Geometry: final body of the model. Coordinates: model frame, mm. A direction names the side the tool comes from. Give positions to 0.01 mm unless a question says otherwise; leave off trailing zeros. Loops run counter-clockwise (first coordinate to the right, second up) from the corner with the lowest first, then second, coordinate; pieces in that order, holes last. Notation, with made-up numbers: (3.5, 22.25) - (10.5, 22.25) arc R22 ccw to (10.5, 35.25) - close; hole circle Ø10 at (52, 49.25). An arc over 180 degrees is marked (long way). Use CSV: the item, a comma, the result in double quotes. Start each with the question number.
```python
from build123d import *

# Parameters (mm, degrees)
SKETCH_1_W          = 50
SKETCH_1_H          = 30
SKETCH_1_W_2        = 44
SKETCH_1_H_2        = 24
EXTRUDE_1_DEPTH     = 450
CUT_EXTRUDE_2_DEPTH = 450
CUT_EXTRUDE_3_DEPTH = 450


with BuildPart() as part:
    # 草图1 → 凸台-拉伸1 (new body)
    with BuildSketch(Plane.XY):
        with Locations((25, 15)):
            Rectangle(SKETCH_1_W, SKETCH_1_H)
        with Locations((25, 15)):
            Rectangle(SKETCH_1_W_2, SKETCH_1_H_2, mode=Mode.SUBTRACT)
    extrude(amount=EXTRUDE_1_DEPTH)

    # 草图2 → 切除-拉伸2 (cut)
    with BuildSketch(Plane.XZ):
        with BuildLine():
            Line((17.5, 430), (17.5, 405))
            ThreePointArc((17.5, 405), (25, 397.5), (32.5, 405))
            Line((32.5, 405), (32.5, 430))
            ThreePointArc((32.5, 430), (25, 437.5), (17.5, 430))
        make_face()
    extrude(amount=-CUT_EXTRUDE_2_DEPTH, mode=Mode.SUBTRACT)

    # 草图4 → 切除-拉伸3 (cut)
    with BuildSketch(Plane.XZ):
        with BuildLine():
            Line((17.5, 380), (17.5, 355))
            ThreePointArc((17.5, 355), (25, 347.5), (32.5, 355))
            Line((32.5, 355), (32.5, 380))
            ThreePointArc((32.5, 380), (25, 387.5), (17.5, 380))
        make_face()
    extrude(amount=-CUT_EXTRUDE_3_DEPTH, mode=Mode.SUBTRACT)


solid = part.part
```
Item 1: Section D-D (z = 413). Output: boundary loops of the cut face in (x, y), plus the area to 3 significant figures.
Item 2: Ray query, probe 1 along Y at (x, z) = (31.5, 141); probe 2 along X at (y, z) = (5, 72.5); probe 3 along X at (y, z) = (2.5, 368). Return the intervals inside material, ascending.
Item 3: Reachability of faces 1 (the cylindrical face through (25.16, 28.48, 387.5)), 2 (the flat face through (3, 15, 222)), 3 (the flat face through (25, 30, 222)) from +Z, -Z, +X, -X, +Y, -Y: full face, straight path, thin tool, end or side. Return the list, or none.
Item 4: Mould query, pull axis Y, two halves, no side actions, for faces 4 (the flat face through (25, 27, 222)), 5 (the flat face through (25, 0, 222)), 6 (the cylindrical face through (24.84, 28.48, 397.5)). Classes: pulls with the +Y half, pulls with the -Y half, needs draft (parallel to the pull), parting line crosses it, or undercut.
Item 5: Section A-A (x = 7). Output: boundary loops of the cut face in (y, z).
Item 6: Section B-B (x = 25). Output: boundary loops of the cut face in (y, z), plus the area to 3 significant figures.
Item 7: Section C-C (z = 314.5). Output: boundary loops of the cut face in (x, y).
Outcome:
1,outline,"(0, 0) - (17.5, 0) - (17.5, 3) - (3, 3) - (3, 27) - (17.5, 27) - (17.5, 30) - (0, 30) - close; (32.5, 0) - (50, 0) - (50, 30) - (32.5, 30) - (32.5, 27) - (47, 27) - (47, 3) - (32.5, 3) - close"
1,area,"354 mm2"
2,probe 1,"y = 0 to 3, 27 to 30"
2,probe 2,"x = 0 to 3, 47 to 50"
2,probe 3,"x = 0 to 17.5, 32.5 to 50"
3,face 1,"+Y, -Y"
3,face 2,"+Z, -Z"
3,face 3,"+Z, -Z, +X, -X, +Y"
4,face 4,"undercut"
4,face 5,"pulls with the -Y half"
4,face 6,"needs draft"
5,outline,"(0, 0) - (3, 0) - (3, 450) - (0, 450) - close; (27, 0) - (30, 0) - (30, 450) - (27, 450) - close"
6,outline,"(0, 0) - (3, 0) - (3, 347.5) - (0, 347.5) - close; (0, 387.5) - (3, 387.5) - (3, 397.5) - (0, 397.5) - close; (0, 437.5) - (3, 437.5) - (3, 450) - (0, 450) - close; (27, 0) - (30, 0) - (30, 347.5) - (27, 347.5) - close; (27, 387.5) - (30, 387.5) - (30, 397.5) - (27, 397.5) - close; (27, 437.5) - (30, 437.5) - (30, 450) - (27, 450) - close"
6,area,"2,220 mm2"
7,outline,"(0, 0) - (50, 0) - (50, 30) - (0, 30) - close; hole (3, 3) - (47, 3) - (47, 27) - (3, 27) - close"
